Read the model definition and answer for the solid it produces. Units are mm, in the model's axes. A direction names the side the tool comes from. Coordinates: 2 decimals unless noted, no trailing zeros. Write each loop counter-clockwise with the first axis right and the second up, starting at its lowest first coordinate (ties: lowest second). Pieces come first, ordered by that corner, then holes. Notation, with made-up numbers: (29, 88) -> (61, 88) arc R22 cw to (61, 122) -> close; hole circle Ø8 at (59.5, -12). An arc over 180 degrees is marked (long way). Answer in a Markdown table with one row per item. Add a question column.
Item 1: Which of the six approach directions +Z, -Z, +X, -X, +Y, -Y give full straight-line access (tool end or side, diameter ignored) to faces 4 (the face through (34.656, -5.89, 7.696)), 5 (the face through (-16.3, -13, 36.3)), 6 (the face through (39.147, -13.986, 18.504))?
Item 2: Section A-A on x = 0 is taken. Write down the section's boundary in (y, z), then the cut area to 3 significant figures.
Item 3: Section C-C on y = -2.75 is taken. Write down the section's boundary in (x, z).
Item 4: Straight lines are drawn through the part: line 1 (X direction, y = -14.2, z = -22.5); line 2 (X direction, y = -13.6, z = 22.5); line 3 (Y direction, x = -3, z = 3). For each, find the intervals that lie inside material, in ascending order. Write a range as from..to.
Item 5: Section D-D on z = 22.5 is taken. Count the separate pieces of the cut face and the enclosed holes in it, then the cut area to 3 significant figures.
Item 6: For a pull along X with two mould halves and no side action, classify faces 1 (the face through (-2.4, -14, -48.2)), 2 (the face through (12, -15, 36)), 3 (the face through (33.27, -4.7, -17.3)) as +X half, -X half, draft (parallel to the pull), parting line (faces both ways), or undercut.
Item 7: Section B-B on z = 45 is taken. Write down the section's boundary in (x, y), then the cut area to 3 significant figures.
Item 8: Given pin 1 Ø8 at (x, y) = (-22.5, 4) entering from +Z; pin 2 Ø6 at (y, z) = (5.5, -29.5) entering from -X; pin 3 Ø6.5 at (x, z) = (38.97, -22.5) entering from -Y; pin 4 Ø9 at (x, z) = (-38.97, 22.5) entering from +Y, each flat-ended and moving along its own axis, determine where each tip first touches the part or whether it passes through.
```python
from build123d import *

# Parameters (mm, degrees)
SKETCH_2_R          = 4
CUT_EXTRUDE_1_DEPTH = 10


with BuildPart() as part:
    # 草图1 → 旋转1 (revolve)
    with BuildSketch(Plane.XY, mode=Mode.PRIVATE) as revolve_1_sk:
        with BuildLine():
            Line((54, -13), (39.5, -13))
            ThreePointArc((39.5, -13), (38.085786438, -12.414213562), (37.5, -11))
            Line((37.5, -11), (37.5, 1.42282291))
            ThreePointArc((37.5, 1.42282291), (33.5233369, 11.0233369), (23.92282291, 15))
            Line((23.92282291, 15), (0, 15))
            Line((0, 15), (0, 13))
            Line((0, 13), (23.92282291, 13))
            ThreePointArc((23.92282291, 13), (32.109123337, 9.609123337), (35.5, 1.42282291))
            Line((35.5, 1.42282291), (35.5, -13))
            ThreePointArc((35.5, -13), (36.085786438, -14.414213562), (37.5, -15))
            Line((37.5, -15), (54, -15))
            Line((54, -15), (54, -13))
        make_face()
    revolve(revolve_1_sk.sketch.rotate(Axis((0, 0, 0), (0, 1, 0)), 90), axis=Axis((0, 0, 0), (0, 1, 0)))

    # 草图2 → 切除-拉伸1 (cut)
    with BuildSketch(Plane(origin=(0, -13, 0), x_dir=(1, 0, 0), z_dir=(0, 1, 0))):
        with Locations(Location((0, 45, 0), (0, 0, 270))):
            Circle(SKETCH_2_R)
        with Locations(Location((38.97114317, 22.5, 0), (0, 0, 270))):
            Circle(SKETCH_2_R)
        with Locations(Location((38.97114317, -22.5, 0), (0, 0, 270))):
            Circle(SKETCH_2_R)
        with Locations(Location((0, -45, 0), (0, 0, 270))):
            Circle(SKETCH_2_R)
        with Locations(Location((-38.97114317, -22.5, 0), (0, 0, 270))):
            Circle(SKETCH_2_R)
        with Locations(Location((-38.97114317, 22.5, 0), (0, 0, 270))):
            Circle(SKETCH_2_R)
    extrude(amount=-CUT_EXTRUDE_1_DEPTH, mode=Mode.SUBTRACT)


solid = part.part
```
Results below:
| question | item | result |
|---|---|---|
| 1 | face 4 | -Y |
| 1 | face 5 | +Y |
| 1 | face 6 | +Y, -Y |
| 2 | outline | (-15, -54) -> (-13, -54) -> (-13, -49) -> (-15, -49) -> close; (-15, -41) -> (-13, -41) -> (-13, -39.5) arc R2 cw to (-11, -37.5) -> (1.42, -37.5) arc R13.58 ccw to (15, -23.92) -> (15, 23.92) arc R13.58 ccw to (1.42, 37.5) -> (-11, 37.5) arc R2 cw to (-13, 39.5) -> (-13, 41) -> (-15, 41) -> (-15, 37.5) arc R2 ccw to (-13, 35.5) -> (1.42, 35.5) arc R11.58 cw to (13, 23.92) -> (13, -23.92) arc R11.58 cw to (1.42, -35.5) -> (-13, -35.5) arc R2 ccw to (-15, -37.5) -> close; (-15, 49) -> (-13, 49) -> (-13, 54) -> (-15, 54) -> close |
| 2 | area | 274 mm2 |
| 3 | outline | circle Ø75 at (0, 0); hole circle Ø71 at (0, 0) |
| 4 | line 1 | x = -49.09..-42.97, -34.97..-27.97, 27.97..34.97, 42.97..49.09 |
| 4 | line 2 | x = -49.09..-42.97, -34.97..-27.58, 27.58..34.97, 42.97..49.09 |
| 4 | line 3 | y = 13..15 |
| 5 | separate pieces | 3 |
| 5 | enclosed holes | 0 |
| 5 | area | 281 mm2 |
| 6 | face 1 | undercut |
| 6 | face 2 | draft |
| 6 | face 3 | parting line |
| 7 | outline | (-29.85, -15) -> (-4, -15) -> (-4, -13) -> (-29.85, -13) -> close; (4, -15) -> (29.85, -15) -> (29.85, -13) -> (4, -13) -> close |
| 7 | area | 103 mm2 |
| 8 | pin 1 | stops at z = 32.44 |
| 8 | pin 2 | stops at x = -25.86 |
| 8 | pin 3 | passes through |
| 8 | pin 4 | stops at y = -13 |
